Geometry: final body of the model. Coordinates: model frame, mm. A direction names the side the tool comes from. Coordinates: 2 decimals unless noted, no trailing zeros. Loops run counter-clockwise (first coordinate to the right, second up) from the corner with the lowest first, then second, coordinate; pieces in that order, holes last. Notation, with made-up numbers: (-0.5, 12.25) -> (36.5, 12.25) arc R23 ccw to (36.5, 45.25) -> close; hole circle Ø4 at (13.5, 11.5). An arc over 180 degrees is marked (long way). One line per item, written item: value. Start each with the question number.
Item 1: Section query A-A on z = 5. Return loops of the section in (x, y).
Item 2: Ray query, probe 1 along Z at (x, y) = (32, 6); probe 2 along Y at (x, z) = (-89.5, 21); probe 3 along X at (y, z) = (6.25, 22.5). Return the intervals inside material, ascending. Write a range as from..to.
Item 3: Section query D-D on y = -22. Return loops of the section in (x, z), then the cut area to 3 significant figures.
Item 4: Section query C-C on x = -85.5. Return loops of the section in (y, z), then the cut area to 3 significant figures.
Item 5: Contact query for flat-ended pins moving along their axis: pin 1 Ø12 at (x, z) = (-60, 19) entering from +Y; pin 2 Ø6.5 at (x, z) = (-102.5, 20.5) entering from +Y; pin 3 Ø2 at (x, z) = (-67, 5.5) entering from -Y. Output: stop coordinate, or through.
Item 6: Section query B-B on x = -125. Return loops of the section in (y, z).
Item 7: Set-up query: faces 5 (the flat face through (-115, -8, 11)), 6 (the flat face through (-114, 12, 22)), 7 (the cylindrical face through (-72.504, 0.385, 18.958)). Return all of +Z, -Z, +X, -X, +Y, -Y with unobstructed straight access to the full face (end or side cutting, diameter ignored); none if empty.
Item 8: Mould query, pull axis Z, two halves, no side actions, for faces 1 (the cylindrical face through (43.997, -5.93, 22.236)), 2 (the cylindrical face through (29, -6.1, 18.5)), 3 (the flat face through (26, 1, 23)), 4 (the flat face through (28, -6, 34.5)). Classes: +Z half, -Z half, draft (parallel to the pull), parting line (faces both ways), or undercut.
from build123d import *

# Parameters (mm, degrees)
HUB_PROFILE_SKETCH_R       = 25
HUB_PROFILE_SKETCH_R_2     = 15
SHAFT_HUB_50_BORE_30_DEPTH = 45
SLOTTED_ARM_END_DEPTH      = 22
ARM_WEB_DEPTH              = 16
CLAMP_LUG_SKETCH_R         = 5
CLAMP_LUG_DEPTH            = 11
CLAMP_SLIT_1MM_DEPTH       = 166.699275798


with BuildPart() as part:
    # Hub Profile Sketch → Shaft Hub Ø50 Bore Ø30 (new body)
    with BuildSketch(Plane.XY):
        with Locations(Location((0, 0, 0), (0, 0, 180))):
            Circle(HUB_PROFILE_SKETCH_R)
        with Locations(Location((0, 0, 0), (0, 0, 180))):
            Circle(HUB_PROFILE_SKETCH_R_2, mode=Mode.SUBTRACT)
    extrude(amount=SHAFT_HUB_50_BORE_30_DEPTH)



with BuildPart() as body_2:
    # Slotted End Sketch → Slotted Arm End (new body)
    with BuildSketch(Plane.XY):
        with BuildLine():
            Line((-140, 17.5), (-90, 17.5))
            ThreePointArc((-90, 17.5), (-72.5, 0), (-90, -17.5))
            Line((-90, -17.5), (-140, -17.5))
            ThreePointArc((-140, -17.5), (-157.5, 0), (-140, 17.5))
        make_face()
        with BuildLine():
            Line((-140, 8), (-90, 8))
            ThreePointArc((-90, 8), (-82, 0), (-90, -8))
            Line((-90, -8), (-140, -8))
            ThreePointArc((-140, -8), (-148, 0), (-140, 8))
        make_face(mode=Mode.SUBTRACT)
    extrude(amount=SLOTTED_ARM_END_DEPTH)


with BuildPart() as part_1:
    add(part.part)

    add(body_2.part)  # Arm Web merges body 2
    # Arm Web Sketch → Arm Web (add)
    with BuildSketch(Plane.XY):
        with BuildLine():
            Line((-1.3438035, 24.963857718), (-140, 17.5))
            Line((-140, 17.5), (-90, 17.5))
            ThreePointArc((-90, 17.5), (-72.5, 0), (-90, -17.5))
            Line((-90, -17.5), (-140, -17.5))
            Line((-140, -17.5), (-2.6709062, -24.856915739))
            ThreePointArc((-2.6709062, -24.856915739), (-24.991135237, 0.665702292), (-1.3438035, 24.963857718))
        make_face()
    extrude(amount=ARM_WEB_DEPTH)

    # Clamp Lug Sketch → Clamp Lug (add, symmetric)
    with BuildSketch(Plane(origin=(0, 0, 0), x_dir=(1, 0, 0), z_dir=(0, 1, 0))):
        with BuildLine():
            Line((32, -34.5), (25, -34.5))
            Line((25, -34.5), (16.676799829, -34.5))
            Line((16.676799829, -34.5), (16.676799829, -10.5))
            Line((16.676799829, -10.5), (25, -10.5))
            Line((25, -10.5), (32, -10.5))
            ThreePointArc((32, -10.5), (44, -22.5), (32, -34.5))
        make_face()
        with Locations(Location((32, -22.5, 0), (0, 0, 270))):
            Circle(CLAMP_LUG_SKETCH_R, mode=Mode.SUBTRACT)
    extrude(amount=CLAMP_LUG_DEPTH, both=True)

    # Clamp Slit Sketch → Clamp Slit 1mm (cut, through all)
    with BuildSketch(Plane.XY.offset(45)):
        with BuildLine():
            Line((14.966629547, -1), (44, -1))
            Line((44, -1), (47.131344101, -1))
            Line((47.131344101, -1), (47.131344101, 1))
            Line((47.131344101, 1), (43.927311634, 1))
            Line((43.927311634, 1), (14.966629547, 1))
            ThreePointArc((14.966629547, 1), (15, 0), (14.966629547, -1))
        make_face()
    extrude(amount=-CLAMP_SLIT_1MM_DEPTH, mode=Mode.SUBTRACT)


solid = part_1.part
Reply:
1. outline: (-140, -17.5) -> (-2.67, -24.86) arc R25 ccw to (24.98, -1) -> (14.97, -1) arc R15 cw (long way) to (14.97, 1) -> (24.98, 1) arc R25 ccw to (-1.34, 24.96) -> (-140, 17.5) arc R17.5 ccw to start; hole (-140, -8) -> (-90, -8) arc R8 ccw to (-90, 8) -> (-140, 8) arc R8 ccw to start
2. probe 1: z = 10.5..17.5, 27.5..34.5
2. probe 2: y = -17.49..-7.98, 7.98..17.49
2. probe 3: x = -24.21..-13.64, 13.64..27, 37..44
3. outline: (-56, 0) -> (11.87, 0) -> (11.87, 45) -> (-11.87, 45) -> (-11.87, 16) -> (-56, 16) -> close
3. area: 1,770 mm²
4. outline: (-20.42, 0) -> (-6.61, 0) -> (-6.61, 22) -> (-16.91, 22) -> (-16.91, 16) -> (-20.42, 16) -> close; (6.61, 0) -> (20.43, 0) -> (20.43, 16) -> (16.91, 16) -> (16.91, 22) -> (6.61, 22) -> close
4. area: 566 mm²
5. pin 1: stops at y = 22.09
5. pin 2: stops at y = 17.5
5. pin 3: stops at y = -21.46
6. outline: (-18.3, 0) -> (-8, 0) -> (-8, 22) -> (-17.5, 22) -> (-17.5, 16) -> (-18.3, 16) -> close; (8, 0) -> (18.31, 0) -> (18.31, 16) -> (17.5, 16) -> (17.5, 22) -> (8, 22) -> close
7. face 5: +Z, -Z
7. face 6: +Z, -X, +Y, -Y
7. face 7: +Z
8. face 1: parting line
8. face 2: undercut
8. face 3: draft
8. face 4: +Z half
